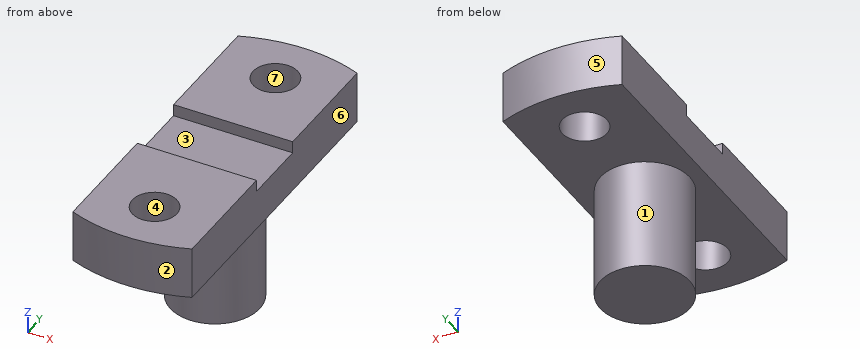
from build123d import *

# Parameters (mm, degrees)
PLATE_PROFILE_SKETCH_R    = 15
KEEPER_PLATE_BODY_DEPTH   = 17.5
MOUNTING_HOLES_SKETCH_W   = 8
MOUNTING_HOLES_SKETCH_H   = 45
MOUNTING_HOLES_DEPTH      = 80
BOSS_60_SKETCH_R          = 30
CYLINDRICAL_BOSS_60_DEPTH = 75


with BuildPart() as part:
    # Plate Profile Sketch → Keeper Plate Body (new, symmetric)
    with BuildSketch(Plane.XY):
        with BuildLine():
            Line((-40, -102.46950766), (-40, 102.46950766))
            ThreePointArc((-40, 102.46950766), (0, 110), (40, 102.46950766))
            Line((40, 102.46950766), (40, -102.46950766))
            ThreePointArc((40, -102.46950766), (0, -110), (-40, -102.46950766))
        make_face()
        with Locations((0, 75)):
            Circle(PLATE_PROFILE_SKETCH_R, mode=Mode.SUBTRACT)
        with Locations(Location((0, -75, 0), (0, 0, 180))):
            Circle(PLATE_PROFILE_SKETCH_R, mode=Mode.SUBTRACT)
    extrude(amount=KEEPER_PLATE_BODY_DEPTH, both=True)

    # Mounting Holes Sketch → Mounting Holes (cut)
    with BuildSketch(Plane(origin=(40, 0, 0), x_dir=(0, 0, -1), z_dir=(1, 0, 0))):
        with Locations((-13.5, 0)):
            Rectangle(MOUNTING_HOLES_SKETCH_W, MOUNTING_HOLES_SKETCH_H)
    extrude(amount=-MOUNTING_HOLES_DEPTH, mode=Mode.SUBTRACT)

    # Boss Ø60 Sketch → Cylindrical Boss Ø60 (add)
    with BuildSketch(Plane(origin=(0, 0, -17.5), x_dir=(-1, 0, 0), z_dir=(0, 0, -1))):
        Circle(BOSS_60_SKETCH_R)
    extrude(amount=CYLINDRICAL_BOSS_60_DEPTH)


solid = part.part
Input: part model. Units: mm. Frame: model coordinates. Face numbers are marked on the shaded views. A direction names the side the tool comes from. Give positions to 0.01 mm unless a question says otherwise; leave off trailing zeros. Write each loop counter-clockwise with the first axis right and the second up, starting at its lowest first coordinate (ties: lowest second). Pieces come first, ordered by that corner, then holes.
Q1. Section C-C, the plane y = 0. Output: boundary loops of the cut face in (x, z).
Q2. Section A-A, the plane x = 0. Output: boundary loops of the cut face in (y, z).
Q3. First-contact query: P1, Ø1, axis at x = -8, z = 1.5, coming from the -Y side; P2, Ø12, axis at y = -24.5, z = -52, coming from the +X side; P3, Ø8, axis at x = 0, z = -73.5, coming from the -Y side. Flat tips, straight axial feed; report the tip coordinate or a pass-through.
Q4. Pull-direction query (Y, two-part tool) for the marked faces 4, 5, 6 and 7; classes: pulls with the +Y half, pulls with the -Y half, needs draft (parallel to the pull), parting line crosses it, or undercut.
Q5. Set-up query: the marked faces 1, 2 and 3. Return all of +Z, -Z, +X, -X, +Y, -Y with unobstructed straight access to the full face (end or side cutting, diameter ignored); none if empty.
Q6. Section D-D, the plane x = 12.5. Output: boundary loops of the cut face in (y, z), plus the area to 3 significant figures.
Q7. Material intervals for probe 1 along Y at (x, z) = (0, 5); probe 2 along X at (y, z) = (-75, 0.5); probe 3 along Y at (x, z) = (-10.5, 6), sorted ascending.
Q8. Section B-B, the plane y = 75. Output: boundary loops of the cut face in (x, z), plus the area to 3 significant figures.
Filled in:
1. outline: (-40, -17.5) - (-30, -17.5) - (-30, -92.5) - (30, -92.5) - (30, -17.5) - (40, -17.5) - (40, 9.5) - (-40, 9.5) - close
2. outline: (-110, -17.5) - (-90, -17.5) - (-90, 17.5) - (-110, 17.5) - close; (-60, -17.5) - (-30, -17.5) - (-30, -92.5) - (30, -92.5) - (30, -17.5) - (60, -17.5) - (60, 17.5) - (22.5, 17.5) - (22.5, 9.5) - (-22.5, 9.5) - (-22.5, 17.5) - (-60, 17.5) - close; (90, -17.5) - (110, -17.5) - (110, 17.5) - (90, 17.5) - close
3. P1: stops at y = -109.74
3. P2: stops at x = 23.62
3. P3: stops at y = -30
4. face 4: undercut
4. face 5: pulls with the +Y half
4. face 6: needs draft
4. face 7: undercut
5. face 1: -Z
5. face 2: +Z, -Z, -Y
5. face 3: +Z, +X, -X
6. outline: (-109.29, -17.5) - (-83.29, -17.5) - (-83.29, 17.5) - (-109.29, 17.5) - close; (-66.71, -17.5) - (-27.27, -17.5) - (-27.27, -92.5) - (27.27, -92.5) - (27.27, -17.5) - (66.71, -17.5) - (66.71, 17.5) - (22.5, 17.5) - (22.5, 9.5) - (-22.5, 9.5) - (-22.5, 17.5) - (-66.71, 17.5) - close; (83.29, -17.5) - (109.29, -17.5) - (109.29, 17.5) - (83.29, 17.5) - close
6. area: 10,200 mm2
7. probe 1: y = -110 to -90, -60 to 60, 90 to 110
7. probe 2: x = -40 to -15, 15 to 40
7. probe 3: y = -109.5 to -85.71, -64.29 to 64.29, 85.71 to 109.5
8. outline: (-40, -17.5) - (-15, -17.5) - (-15, 17.5) - (-40, 17.5) - close; (15, -17.5) - (40, -17.5) - (40, 17.5) - (15, 17.5) - close
8. area: 1,750 mm2
